```python
from build123d import *

# Parameters (mm, degrees)
SKETCH1_W           = 300
SKETCH1_H           = 370
SKETCH1_R           = 13.75
BOSS_EXTRUDE1_DEPTH = 25


with BuildPart() as part:
    # Sketch1 → Boss-Extrude1 (new body)
    with BuildSketch(Plane.XY):
        with Locations((150, 185)):
            Rectangle(SKETCH1_W, SKETCH1_H)
        with Locations((225, 305)):
            Circle(SKETCH1_R, mode=Mode.SUBTRACT)
        with Locations((225, 185)):
            Circle(SKETCH1_R, mode=Mode.SUBTRACT)
        with Locations((225, 65)):
            Circle(SKETCH1_R, mode=Mode.SUBTRACT)
    extrude(amount=BOSS_EXTRUDE1_DEPTH)


solid = part.part
```
Input: part model. Units: mm. Frame: model coordinates. Give positions to 0.01 mm unless a question says otherwise; leave off trailing zeros. Order: outer loops, then holes, each group sorted by start corner. A loop starts at its lowest first (then second) coordinate and runs counter-clockwise, first axis right, second up.
1. Material intervals for L1, parallel to X at y = 180, z = 14.25; L2, parallel to X at y = 178.5, z = 5.5, sorted ascending.
Derived:
L1: x = 0 to 212.19, 237.81 to 300
L2: x = 0 to 212.88, 237.12 to 300
2. Section B-B on z = 7.75. Return the cut outline in (x, y).
Derived:
outline: (0, 0) - (300, 0) - (300, 370) - (0, 370) - close; hole circle Ø27.5 at (225, 65); hole circle Ø27.5 at (225, 185); hole circle Ø27.5 at (225, 305)
3. Section C-C on y = 65. Return the cut outline in (x, z).
Derived:
outline: (0, 0) - (211.25, 0) - (211.25, 25) - (0, 25) - close; (238.75, 0) - (300, 0) - (300, 25) - (238.75, 25) - close
4. Section D-D on y = 181. Return the cut outline in (x, z), and give its area (3 significant figures).
Derived:
outline: (0, 0) - (211.84, 0) - (211.84, 25) - (0, 25) - close; (238.16, 0) - (300, 0) - (300, 25) - (238.16, 25) - close
area: 6,840 mm2
5. Section A-A on x = 225. Return the cut outline in (y, z), and give its area (3 significant figures).
Derived:
outline: (0, 0) - (51.25, 0) - (51.25, 25) - (0, 25) - close; (78.75, 0) - (171.25, 0) - (171.25, 25) - (78.75, 25) - close; (198.75, 0) - (291.25, 0) - (291.25, 25) - (198.75, 25) - close; (318.75, 0) - (370, 0) - (370, 25) - (318.75, 25) - close
area: 7,190 mm2
6. Pin query (flat end, axial travel): pin 1 (22 mm diameter, centred on x = 225, y = 305, fed in from -Z). Return the tip coordinate at first contact, or that it passes through.
Derived:
pin 1: passes through
7. Mould query, pull axis X, two halves, no side actions, for faces 1 (the cylindrical face through (237.7, 179.73, 12.32)), 2 (the flat face through (148, 370, 12)), 3 (the flat face through (0, 182, 12)). Classes: released by +X, released by -X, zero draft, split by the parting line, or undercut.
Derived:
face 1: undercut
face 2: zero draft
face 3: released by -X
